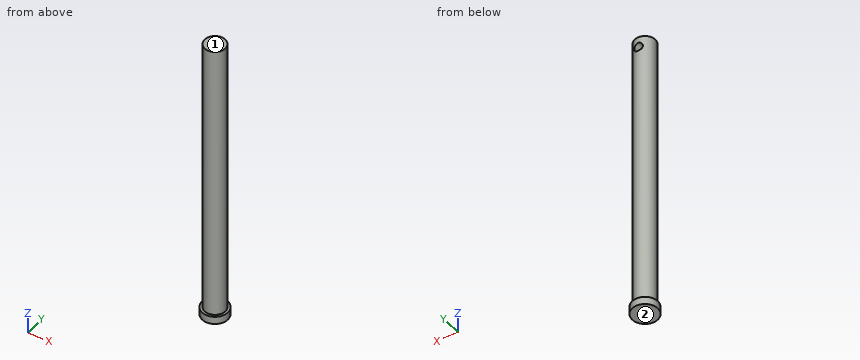
from build123d import *

# Parameters (mm, degrees)
SKETCH1_R           = 4
BOSS_EXTRUDE1_DEPTH = 110
SKETCH7_R           = 5
BOSS_EXTRUDE2_DEPTH = 3
SKETCH9_W           = 1.65
SKETCH9_H           = 5


with BuildPart() as part:
    # Sketch1 → Boss-Extrude1 (new body)
    with BuildSketch(Plane.XY):
        Circle(SKETCH1_R)
    extrude(amount=BOSS_EXTRUDE1_DEPTH)

    # Sketch7 → Boss-Extrude2 (add)
    with BuildSketch(Plane(origin=(0, 0, 0), x_dir=(-1, 0, 0), z_dir=(0, 0, -1))):
        Circle(SKETCH7_R)
    extrude(amount=BOSS_EXTRUDE2_DEPTH)

    # Sketch9 → M4 Tapped Hole1 (revolve, cut)
    with BuildSketch(Plane(origin=(0, 0, 106), x_dir=(0, 0, -1), z_dir=(1, 0, 0))):
        with Locations((0.825, 2.5)):
            Rectangle(SKETCH9_W, SKETCH9_H)
    revolve(axis=Axis((0, -6.35, 106), (0, 1, 0)), mode=Mode.SUBTRACT)


solid = part.part
Work out the finished part from the listing and answer in its coordinate system (mm). Face numbers are marked on the shaded views. Round coordinates to 2 decimals unless told otherwise and drop trailing zeros. Order: outer loops, then holes, each group sorted by start corner. A loop starts at its lowest first (then second) coordinate and runs counter-clockwise, first axis right, second up. Notation, with made-up numbers: M -36.5,65.25 L -19.5,65.25 A14 ccw -19.5,71.25 Z; hole C -29.5,-0.5 d9. An arc over 180 degrees is marked long. One line per item, written item: value.
Q1. Flat-ended cylindrical pins translate along their axes: pin 1 (6 mm diameter, centred on x = -0.5, z = 24, fed in from -Y); pin 2 (2 mm diameter, centred on y = -2.5, z = 74, fed in from -X); pin 3 (1 mm diameter, centred on x = 0, z = 106, fed in from +Y). Find the tip coordinate at first contact, or state that the pin passes through.
Derived:
pin 1: y = -4
pin 2: x = -3.71
pin 3: y = 0
Q2. Straight lines are drawn through the part: line 1 (Z direction, x = 0, y = 1.4); line 2 (Z direction, x = 4.5, y = -2); line 3 (X direction, y = 1.65, z = 106). For each, find the intervals that lie inside material, in ascending order.
Derived:
line 1: -3 to 104.35, 107.65 to 110
line 2: -3 to 0
line 3: -3.64 to -1.65, 1.65 to 3.64
Q3. Determine the mould class of the marked faces 1 and 2 for opening direction Z: released by +Z, released by -Z, zero draft, split by the parting line, or undercut.
Derived:
face 1: released by +Z
face 2: released by -Z
Q4. Find section C-C on z = 90. Write down the section's boundary in (x, y).
Derived:
outline: C 0,0 d8
Q5. Find section A-A on x = 0. Write down the section's boundary in (y, z).
Derived:
outline: M -5,-3 L 5,-3 L 5,0 L 4,0 L 4,104.35 L 0,104.35 L 0,107.65 L 4,107.65 L 4,110 L -4,110 L -4,0 L -5,0 Z
Q6. Find section B-B on y = 2.25. Write down the section's boundary in (x, z), then the cut area to 3 significant figures.
Derived:
outline: M -4.47,-3 L 4.47,-3 L 4.47,0 L 3.31,0 L 3.31,110 L -3.31,110 L -3.31,0 L -4.47,0 Z; hole C 0,106 d3.3
area: 746 mm²
Q7. Find section D-D on z = 106. Write down the section's boundary in (x, y).
Derived:
outline: M -1.65,0 L -1.65,3.64 A4 ccw long 1.65,3.64 L 1.65,0 Z
